The model under review builds one solid part; all positions refer to its coordinate system, in mm. Coordinates: 2 decimals unless noted, no trailing zeros. Order: outer loops, then holes, each group sorted by start corner. A loop starts at its lowest first (then second) coordinate and runs counter-clockwise, first axis right, second up. Notation, with made-up numbers: M 5,17 L 42,17 A24 cw 42,48 Z; hole C -29,51.25 d1. An arc over 180 degrees is marked long. Answer in a Markdown table with one row per item.
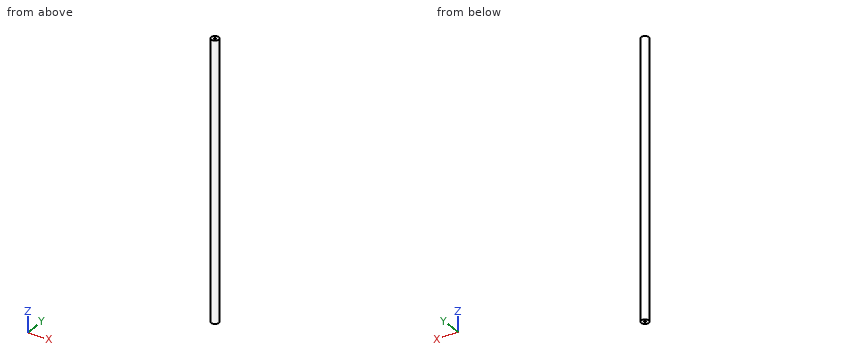
from build123d import *

# Parameters (mm, degrees)
SKETCH_1_R             = 6
EXTRUDE_1_DEPTH        = 448
HOLE_WIZARD_M4_1_D     = 3.3
HOLE_WIZARD_M4_1_DEPTH = 15
HOLE_WIZARD_M4_1_TIP   = 0.991420021
HOLE_WIZARD_M4_2_D     = 3.3
HOLE_WIZARD_M4_2_DEPTH = 15
HOLE_WIZARD_M4_2_TIP   = 0.991420021


with BuildPart() as part:
    # 草图1 → 凸台-拉伸1 (new body)
    with BuildSketch(Plane.XY):
        Circle(SKETCH_1_R)
    extrude(amount=EXTRUDE_1_DEPTH)

    # M4 螺纹孔1
    with Locations(Plane(origin=(0, 0, 0), x_dir=(-1, 0, 0), z_dir=(0, 0, -1))):
        with Locations((0, 0)):
            Hole(HOLE_WIZARD_M4_1_D / 2, depth=HOLE_WIZARD_M4_1_DEPTH)
            with Locations((0, 0, -(HOLE_WIZARD_M4_1_DEPTH + HOLE_WIZARD_M4_1_TIP / 2))):  # 118° drill point
                Cone(0, HOLE_WIZARD_M4_1_D / 2, HOLE_WIZARD_M4_1_TIP, mode=Mode.SUBTRACT)

    # M4 螺纹孔2
    with Locations(Plane.XY.offset(448)):
        with Locations((0, 0)):
            Hole(HOLE_WIZARD_M4_2_D / 2, depth=HOLE_WIZARD_M4_2_DEPTH)
            with Locations((0, 0, -(HOLE_WIZARD_M4_2_DEPTH + HOLE_WIZARD_M4_2_TIP / 2))):  # 118° drill point
                Cone(0, HOLE_WIZARD_M4_2_D / 2, HOLE_WIZARD_M4_2_TIP, mode=Mode.SUBTRACT)


solid = part.part
(1) Take a section at A-A (z = 337). Write out the cut boundary in (x, y), then the cut area to 3 significant figures.
Report:
| item | result |
|---|---|
| outline | C 0,0 d12 |
| area | 113 mm^2 |
(2) To check wall thickness, follow line 1 (Y direction, x = 0, z = 5.75); line 2 (X direction, y = -0.5, z = 396); line 3 (X direction, y = 2.75, z = 229). State the ranges of each line that lie inside material, in increasing order. Write a range as [from, to].
Report:
| item | result |
|---|---|
| line 1 | [-6, -1.65], [1.65, 6] |
| line 2 | [-5.98, 5.98] |
| line 3 | [-5.33, 5.33] |
(3) Take a section at B-B (x = 4). Write out the cut boundary in (y, z), then the cut area to 3 significant figures.
Report:
| item | result |
|---|---|
| outline | M -4.47,0 L 4.47,0 L 4.47,448 L -4.47,448 Z |
| area | 4,010 mm^2 |
(4) Insertion check: P1, Ø1, axis at x = 1.5, z = 150, coming from the -Y side; P2, Ø1, axis at x = -4.5, y = 3, coming from the -Z side; P3, Ø5, axis at x = 4, z = 385.5, coming from the +Y side; P4, Ø4, axis at y = 2.5, z = 236.5, coming from the +X side. Each pin has a flat end and moves straight along its axis. Give the tip position at first contact, or say it passes through.
Report:
| item | result |
|---|---|
| P1 | y = -5.92 |
| P2 | z = 0 |
| P3 | y = 5.81 |
| P4 | x = 5.98 |
(5) Take a section at C-C (y = -3.5). Write out the cut boundary in (x, z), then the cut area to 3 significant figures.
Report:
| item | result |
|---|---|
| outline | M -4.87,0 L 4.87,0 L 4.87,448 L -4.87,448 Z |
| area | 4,370 mm^2 |
